Could you check a few things on this model? Use its own coordinates, in mm. A direction names the side the tool comes from. Give positions to 0.01 mm unless a question says otherwise; leave off trailing zeros. Order: outer loops, then holes, each group sorted by start corner. A loop starts at its lowest first (then second) coordinate and runs counter-clockwise, first axis right, second up. Notation, with made-up numbers: M -12.5,58 L 35.5,58 A22 ccw 35.5,94 Z; hole C -14.5,33.5 d1. An arc over 180 degrees is marked long. Return JSON: item names as keys, results as strings. Group by question number.
```python
from build123d import *

# Parameters (mm, degrees)
SKETCH1_R           = 37.5
SKETCH1_R_2         = 25
BOSS_EXTRUDE1_DEPTH = 15
SKETCH2_R           = 30
CUT_EXTRUDE1_DEPTH  = 5
CUT_EXTRUDE2_DEPTH  = 5
SKETCH4_R           = 1.5
CUT_EXTRUDE3_DEPTH  = 10


with BuildPart() as part:
    # Sketch1 → Boss-Extrude1 (new body)
    with BuildSketch(Plane.XY):
        Circle(SKETCH1_R)
        Circle(SKETCH1_R_2, mode=Mode.SUBTRACT)
    extrude(amount=BOSS_EXTRUDE1_DEPTH)

    # Sketch2 → Cut-Extrude1 (cut)
    with BuildSketch(Plane(origin=(0, 0, 0), x_dir=(-1, 0, 0), z_dir=(0, 0, -1))):
        Circle(SKETCH2_R)
    extrude(amount=-CUT_EXTRUDE1_DEPTH, mode=Mode.SUBTRACT)

    # Sketch3 → Cut-Extrude2 (cut)
    with BuildSketch(Plane(origin=(0, 0, 0), x_dir=(-1, 0, 0), z_dir=(0, 0, -1))):
        with BuildLine():
            Line((0, 30), (0, 37.5))
            ThreePointArc((0, 37.5), (7.315887076, 36.779448015), (14.350628714, 34.645482469))
            Line((14.350628714, 34.645482469), (11.480502971, 27.716385975))
            ThreePointArc((11.480502971, 27.716385975), (5.85270966, 29.423558412), (0, 30))
        make_face()
        with BuildLine():
            Line((21.213203436, 21.213203436), (26.516504294, 26.516504294))
            ThreePointArc((26.516504294, 26.516504294), (31.180110461, 20.833883738), (34.645482469, 14.350628714))
            Line((34.645482469, 14.350628714), (27.716385975, 11.480502971))
            ThreePointArc((27.716385975, 11.480502971), (24.944088369, 16.667106991), (21.213203436, 21.213203436))
        make_face()
        with BuildLine():
            Line((30, 0), (37.5, 0))
            ThreePointArc((37.5, 0), (36.779448015, -7.315887076), (34.645482469, -14.350628714))
            Line((34.645482469, -14.350628714), (27.716385975, -11.480502971))
            ThreePointArc((27.716385975, -11.480502971), (29.423558412, -5.85270966), (30, 0))
        make_face()
        with BuildLine():
            Line((21.213203436, -21.213203436), (26.516504294, -26.516504294))
            ThreePointArc((26.516504294, -26.516504294), (20.833883738, -31.180110461), (14.350628714, -34.645482469))
            Line((14.350628714, -34.645482469), (11.480502971, -27.716385975))
            ThreePointArc((11.480502971, -27.716385975), (16.667106991, -24.944088369), (21.213203436, -21.213203436))
        make_face()
        with BuildLine():
            Line((0, -30), (0, -37.5))
            ThreePointArc((0, -37.5), (-7.315887076, -36.779448015), (-14.350628714, -34.645482469))
            Line((-14.350628714, -34.645482469), (-11.480502971, -27.716385975))
            ThreePointArc((-11.480502971, -27.716385975), (-5.85270966, -29.423558412), (0, -30))
        make_face()
        with BuildLine():
            Line((-21.213203436, -21.213203436), (-26.516504294, -26.516504294))
            ThreePointArc((-26.516504294, -26.516504294), (-31.180110461, -20.833883738), (-34.645482469, -14.350628714))
            Line((-34.645482469, -14.350628714), (-27.716385975, -11.480502971))
            ThreePointArc((-27.716385975, -11.480502971), (-24.944088369, -16.667106991), (-21.213203436, -21.213203436))
        make_face()
        with BuildLine():
            Line((-30, 0), (-37.5, 0))
            ThreePointArc((-37.5, 0), (-36.779448015, 7.315887076), (-34.645482469, 14.350628714))
            Line((-34.645482469, 14.350628714), (-27.716385975, 11.480502971))
            ThreePointArc((-27.716385975, 11.480502971), (-29.423558412, 5.85270966), (-30, 0))
        make_face()
        with BuildLine():
            Line((-21.213203436, 21.213203436), (-26.516504294, 26.516504294))
            ThreePointArc((-26.516504294, 26.516504294), (-20.833883738, 31.180110461), (-14.350628714, 34.645482469))
            Line((-14.350628714, 34.645482469), (-11.480502971, 27.716385975))
            ThreePointArc((-11.480502971, 27.716385975), (-16.667106991, 24.944088369), (-21.213203436, 21.213203436))
        make_face()
    extrude(amount=-CUT_EXTRUDE2_DEPTH, mode=Mode.SUBTRACT)

    # Sketch4 → Cut-Extrude3 (cut)
    with BuildSketch(Plane(origin=(0, 0, 5), x_dir=(-1, 0, 0), z_dir=(0, 0, -1))):
        with Locations((4.960455731, 32.119213548)):
            Circle(SKETCH4_R)
    extrude(amount=-CUT_EXTRUDE3_DEPTH, mode=Mode.SUBTRACT)


solid = part.part
```
1. Imagine slicing it at D-D, the plane z = 12.25. Please give me the cut outline in (x, y).
2. Imagine slicing it at B-B, the plane y = -13. Please give me the cut outline in (x, z), plus the area to 3 significant figures.
3. I need wall thicknesses on L1, parallel to X at y = 0, z = 11.25; L2, parallel to Z at x = 7.5, y = 24.5. Which ranges of each line are inside material? Lowest first, please. Write a range as from..to.
4. Which directions (+Z, -Z, +X, -X, +Y, -Y) give clear straight access to the entire face, cutting with the end or side of a thin tool? Please do faces 4 (the flat face through (-31.229, -12.936, 2.465)), 5 (the flat face through (5, -25, 5)), 6 (the flat face through (24, 24, 2)), 7 (the flat face through (12.936, -31.229, 2.465)), 8 (the cylindrical face through (-4.635, 30.655, 9.93)).
5. If we mould it in two halves opening along X, with no side actions, what happens to faces 1 (the flat face through (0, -34, 2)), 2 (the flat face through (24, -24, 2)), 3 (the flat face through (7, 33, 0))? For each: pulls with the +X half, pulls with the -X half, needs draft (parallel to the pull), parting line crosses it, or undercut.
6. Imagine slicing it at A-A, the plane x = 1. Please give me the cut outline in (y, z).
7. For pin 1 (2.5 mm diameter, centred on y = 32, z = 3, fed in from -X); pin 2 (5 mm diameter, centred on x = 26.5, z = 11, fed in from -Y); pin 3 (2.5 mm diameter, centred on x = -33.5, z = 2.5, fed in from -Y); pin 4 (2.5 mm diameter, centred on x = -4.96, y = 32.12, fed in from -Z), each with a flat end and sliding along its axis, tell me the tip position at first contact or that it passes through.
8. Imagine slicing it at C-C, the plane x = -22.5. Please give me the cut outline in (y, z).
Values:
{
 "1": {"outline": "C 0,0 d75; hole C 0,0 d50; hole C -4.96,32.12 d3"},
 "2": {"outline": "M -35.17,5 L -31.38,5 L -31.38,0 L -27.04,0 L -27.04,5 L -21.35,5 L -21.35,15 L -35.17,15 Z; M 21.35,5 L 31.38,5 L 31.38,0 L 35.17,0 L 35.17,15 L 21.35,15 Z", "area": "317 mm²"},
 "3": {"L1": "x = -37.5..-25, 25..37.5", "L2": "z = 5..15"},
 "4": {"face 4": "-Z, -X", "face 5": "-Z", "face 6": "-Z, +Y", "face 7": "-Z, -Y", "face 8": "+Z, -Z"},
 "5": {"face 1": "undercut", "face 2": "pulls with the +X half", "face 3": "needs draft"},
 "6": {"outline": "M -37.49,5 L -24.98,5 L -24.98,15 L -37.49,15 Z; M 24.98,5 L 29.98,5 L 29.98,0 L 37.49,0 L 37.49,15 L 24.98,15 Z"},
 "7": {"pin 1": "stops at x = -21.46", "pin 2": "stops at y = -28.81", "pin 3": "stops at y = -19.14", "pin 4": "passes through"},
 "8": {"outline": "M -30,5 L -22.5,5 L -22.5,0 L -19.84,0 L -19.84,5 L -10.9,5 L -10.9,15 L -30,15 Z; M 10.9,5 L 22.5,5 L 22.5,0 L 30,0 L 30,15 L 10.9,15 Z"}
}
